Here's the drawing with two shaded views (mm, measured from the low corner). I have some questions. A direction names the side the tool comes from. Coordinates: 2 decimals unless noted, no trailing zeros. Write each loop counter-clockwise with the first axis right and the second up, starting at its lowest first coordinate (ties: lowest second). Pieces come first, ordered by that corner, then holes.
Item 1: If we section it at B-B (x = 10): Please give me the cut outline in (y, z), then the cut area to 3 significant figures.
Item 2: We'd pull the mould along X, two halves only. Please class the marked faces 1, 2 and 3: +X half, -X half, draft (parallel to the pull), parting line (faces both ways), or undercut.
Item 3: If we section it at D-D (x = 18): Please give me the cut outline in (y, z), then the cut area to 3 significant figures.
Item 4: For the marked faces 4, 5 and 6, which set-ups out of +Z, -Z, +X, -X, +Y, -Y let a thin tool reach every point of the face, with its end or its side?
Item 5: If we section it at A-A (y = 27): Please give me the cut outline in (x, z), then the cut area to 3 significant figures.
Item 6: If we section it at C-C (z = 60): Please give me the cut outline in (x, y).
Item 7: I'm going to push flat-ended pins straight in: pin 1 Ø6 at (x, z) = (5.5, 31.5) entering from -Y; pin 2 Ø3.5 at (x, y) = (11.5, 48.5) entering from +Z; pin 3 Ø6 at (x, z) = (14, 29.5) entering from +Y. Where does each tip first touch, or does it pass through?
Item 8: If I drill on line 1 (Y direction, x = 10, z = 6.6); line 2 (Y direction, x = 10, z = 1.6); line 3 (Z direction, x = 17.5, y = 29.5), over which ranges is the centre line in solid material (lowest first)?
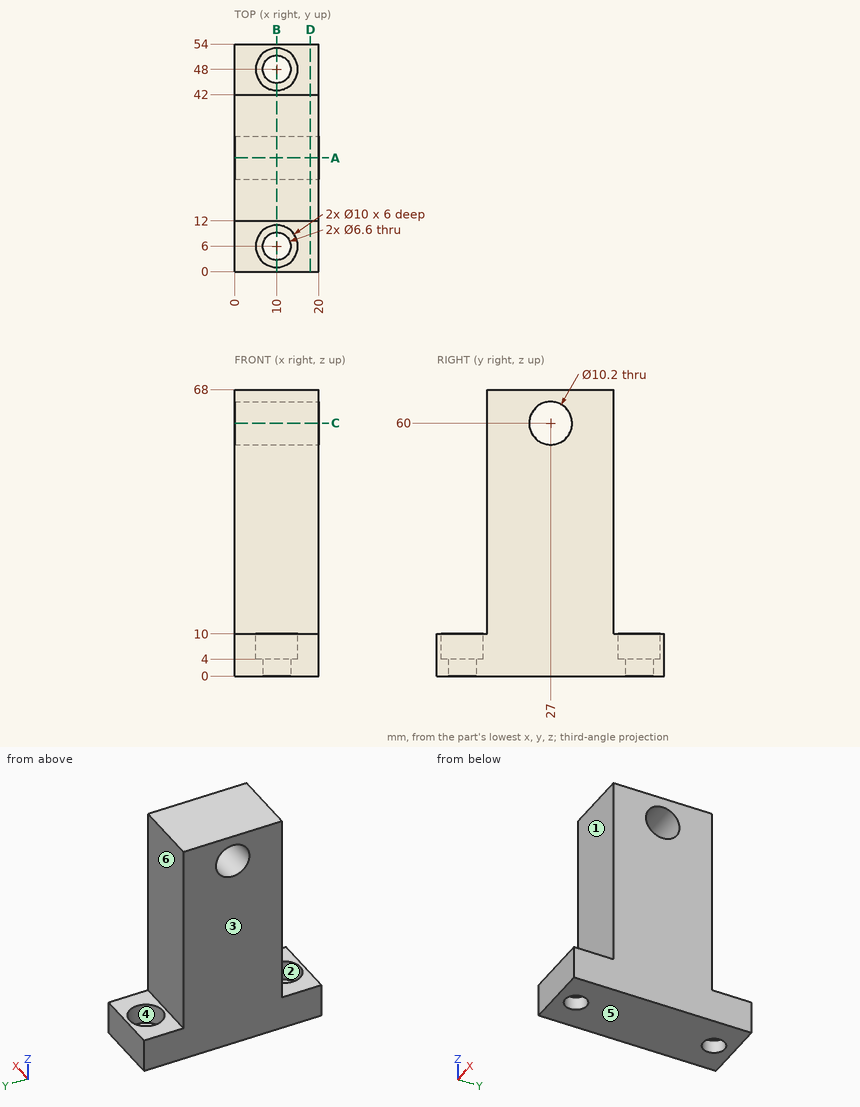
Answer list:
1. outline: (0, 0) - (2.7, 0) - (2.7, 4) - (1, 4) - (1, 10) - (0, 10) - close; (9.3, 0) - (44.7, 0) - (44.7, 4) - (43, 4) - (43, 10) - (42, 10) - (42, 68) - (12, 68) - (12, 10) - (11, 10) - (11, 4) - (9.3, 4) - close; (51.3, 0) - (54, 0) - (54, 10) - (53, 10) - (53, 4) - (51.3, 4) - close; hole circle Ø10.2 at (27, 60)
1. area: 2,030 mm2
2. face 1: draft
2. face 2: undercut
2. face 3: -X half
3. outline: (0, 0) - (54, 0) - (54, 10) - (42, 10) - (42, 68) - (12, 68) - (12, 10) - (0, 10) - close; hole circle Ø10.2 at (27, 60)
3. area: 2,200 mm2
4. face 4: +Z
4. face 5: -Z, +X, -X, +Y, -Y
4. face 6: +Z, +X, -X, +Y
5. outline: (0, 0) - (20, 0) - (20, 54.9) - (0, 54.9) - close; (0, 65.1) - (20, 65.1) - (20, 68) - (0, 68) - close
5. area: 1,160 mm2
6. outline: (0, 12) - (20, 12) - (20, 21.9) - (0, 21.9) - close; (0, 32.1) - (20, 32.1) - (20, 42) - (0, 42) - close
7. pin 1: stops at y = 12
7. pin 2: stops at z = 4
7. pin 3: stops at y = 42
8. line 1: y = 0 to 1, 11 to 43, 53 to 54
8. line 2: y = 0 to 2.7, 9.3 to 44.7, 51.3 to 54
8. line 3: z = 0 to 55.55, 64.45 to 68
